from build123d import *

# Parameters (mm, degrees)
EXTRUDE_2_DEPTH              = 40
SKETCH_4_W                   = 2.5
SKETCH_4_H                   = 90
CUT_EXTRUDE_2_DEPTH          = 80
EXTRUDE_3_DEPTH              = 5
FILLET_1_R                   = 10
CHAMFER_1_SIZE               = 10
HOLE_WIZARD_M6_1_D           = 6.6
HOLE_WIZARD_M6_1_CBORE_D     = 11
HOLE_WIZARD_M6_1_CBORE_DEPTH = 6.4
CHAMFER_2_SIZE               = 3
HOLE_WIZARD_7_0_7_1_D        = 7
HOLE_WIZARD_M8_2_D           = 9
HOLE_WIZARD_M8_2_CBORE_D     = 15
HOLE_WIZARD_M8_2_CBORE_DEPTH = 8.6
SKETCH_16_W                  = 163.711624667
SKETCH_16_H                  = 2.5
CUT_EXTRUDE_3_DEPTH          = 179.955301682
SKETCH_17_W                  = 70
SKETCH_17_H                  = 9
CUT_EXTRUDE_4_DEPTH          = 198.834526815
CHAMFER_4_SIZE               = 3
HOLE_WIZARD_7_0_7_2_D        = 7
HOLE_WIZARD_6_0_6_1_D        = 6


with BuildPart() as part:
    # 草图2 → 凸台-拉伸2 (new, symmetric)
    with BuildSketch(Plane.XY):
        Polygon((46, -8.5), (80, -8.5), (80, 8.5), (72, 8.5), (72, 163.5), (56, 163.5), (56, 8.5), (-80, 8.5), (-80, -8.5), (-2, -8.5), (-2, -6.5), (46, -6.5), align=None)
    extrude(amount=EXTRUDE_2_DEPTH, both=True)

    # 草图4 → 切除-拉伸2 (cut)
    with BuildSketch(Plane.ZY.offset(-56)):
        with Locations((-38.75, 53.5)):
            Rectangle(SKETCH_4_W, SKETCH_4_H)
    extrude(amount=-CUT_EXTRUDE_2_DEPTH, mode=Mode.SUBTRACT)

    # 草图5 → 凸台-拉伸3 (add, symmetric)
    with BuildSketch(Plane.XY):
        Polygon((46, 8.5), (6, 8.5), (6, 26.5), (38, 26.5), (38, 83.5), (56, 83.5), (56, 18.5), align=None)
    extrude(amount=EXTRUDE_3_DEPTH, both=True)

    # 圆角1
    fillet_1_edges = [part.edges().sort_by_distance(p)[0] for p in [
        (38, 26.5, 0),
    ]]
    fillet(fillet_1_edges, radius=FILLET_1_R)

    # 倒角1
    chamfer_1_edges = [part.edges().sort_by_distance(p)[0] for p in [
        (6, 26.5, 0),
        (38, 83.5, 0),
    ]]
    chamfer(chamfer_1_edges, length=CHAMFER_1_SIZE)

    # M6 六角凹头螺钉的柱形沉头孔1 (through all)
    with Locations(Plane(origin=(0, 8.5, 0), x_dir=(1, 0, 0), z_dir=(0, 1, 0))):
        with Locations((4.5, 17.5), (39.5, 17.5), (39.5, -17.5), (4.5, -17.5)):
            CounterBoreHole(HOLE_WIZARD_M6_1_D / 2, HOLE_WIZARD_M6_1_CBORE_D / 2, HOLE_WIZARD_M6_1_CBORE_DEPTH)

    # 倒角2
    chamfer_2_edges = [part.edges().sort_by_distance(p)[0] for p in [
        (64, 163.5, 40),
        (64, 163.5, -40),
        (80, 0, -40),
        (-80, 0, 40),
        (80, 0, 40),
    ]]
    chamfer(chamfer_2_edges, length=CHAMFER_2_SIZE)

    # Ø7.0 (7) 直径孔1 (through all)
    with Locations(Plane.ZY.offset(-56)):
        with Locations((-31, 25.5), (-31, 66.5), (31, 66.5), (31, 25.5)):
            Hole(HOLE_WIZARD_7_0_7_1_D / 2)

    # M8 六角凹头螺钉的柱形沉头孔2 (through all)
    with Locations(Plane.ZY.offset(-56)):
        with Locations((-20, 143.5), (-20, 103.5), (20, 103.5), (20, 143.5)):
            CounterBoreHole(HOLE_WIZARD_M8_2_D / 2, HOLE_WIZARD_M8_2_CBORE_D / 2, HOLE_WIZARD_M8_2_CBORE_DEPTH)

    # 草图16 → 切除-拉伸3 (cut, through all)
    with BuildSketch(Plane(origin=(0, 8.5, 0), x_dir=(1, 0, 0), z_dir=(0, 1, 0))):
        with Locations((-1.855812334, 38.75)):
            Rectangle(SKETCH_16_W, SKETCH_16_H)
    extrude(amount=-CUT_EXTRUDE_3_DEPTH, mode=Mode.SUBTRACT)

    # 草图17 → 切除-拉伸4 (cut, through all)
    with BuildSketch(Plane(origin=(0, 0, -37.5), x_dir=(-1, 0, 0), z_dir=(0, 0, -1))):
        with Locations((45, -4)):
            Rectangle(SKETCH_17_W, SKETCH_17_H)
    extrude(amount=-CUT_EXTRUDE_4_DEPTH, mode=Mode.SUBTRACT)

    # 倒角4
    chamfer_4_edges = [part.edges().sort_by_distance(p)[0] for p in [
        (-80, 4.5, -37.5),
    ]]
    chamfer(chamfer_4_edges, length=CHAMFER_4_SIZE)

    # Ø7.0 (7) 直径孔2 (through all)
    with Locations(Plane(origin=(0, 8.5, 0), x_dir=(1, 0, 0), z_dir=(0, 1, 0))):
        with Locations((-28, 15), (-60, 15)):
            Hole(HOLE_WIZARD_7_0_7_2_D / 2)

    # Ø6.0 (6) 直径孔1 (through all)
    with Locations(Plane(origin=(0, 8.5, 0), x_dir=(1, 0, 0), z_dir=(0, 1, 0))):
        with Locations((-70, -31), (-70, -19)):
            Hole(HOLE_WIZARD_6_0_6_1_D / 2)


solid = part.part
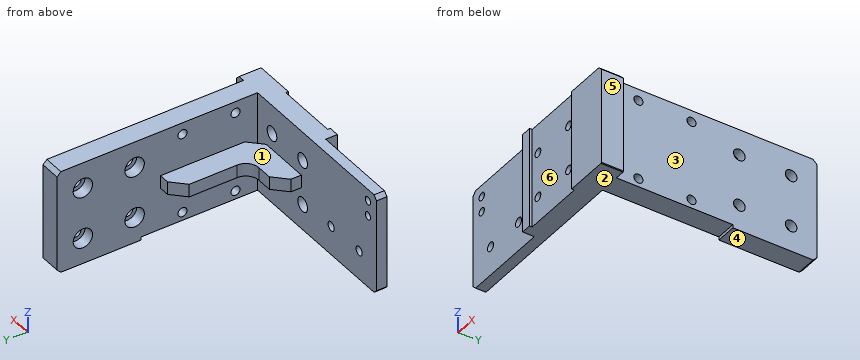
Model file for the job. Use its own axes, mm. Face numbers are marked on the shaded views. A direction names the side the tool comes from. Coordinates: 2 decimals unless noted, no trailing zeros. Order: outer loops, then holes, each group sorted by start corner. A loop starts at its lowest first (then second) coordinate and runs counter-clockwise, first axis right, second up. Notation, with made-up numbers: (-13, 33.5) -> (3, 33.5) arc R5 ccw to (3, 38.5) -> close; hole circle Ø8 at (-2, -2). An arc over 180 degrees is marked (long way). Return JSON: item names as keys, results as strings. Group by question number.
Item 1: Saw through at C-C on z = 31. Write the cut outline in (x, y).
Item 2: Saw through at A-A on x = -70. Write the cut outline in (y, z), then the cut area to 3 significant figures.
Item 3: Wall check: line 1 along Z through (x, y) = (4, 6); line 2 along Y through (x, z) = (58, -20); line 3 along Y through (x, z) = (68.25, -20). Give the ranges that are in metal, low to high. Write a range as [from, to].
Item 4: Saw through at D-D on x = 58.5. State how many separate pieces and enclosed holes the cut face has, then the cut area to 3 significant figures.
Item 5: Flat gauge pins, fed straight in: P1, Ø6.5, axis at x = 51.5, z = 2, coming from the +Y side; P2, Ø2.5, axis at x = 74.5, z = -10, coming from the +Y side; P3, Ø6, axis at y = 80, z = 24, coming from the -X side. Where does each tip first touch, or does it go through?
Item 6: Pull direction X, two halves, no side cores. Call the marked faces 4, 5 and 6: pulls with the +X half, pulls with the -X half, needs draft (parallel to the pull), parting line crosses it, or undercut.
Item 7: Saw through at B-B on y = 103.5. Write the cut outline in (x, z).
Item 8: Tool access for the marked faces 1, 2 and 3: list every direction of +Z, -Z, +X, -X, +Y, -Y with a clear straight run to the whole face (end or side of a thin tool).
Values found:
{
 "1": {"outline": "(-80, 0.5) -> (-73, 0.5) -> (-73, 8.5) -> (-80, 8.5) -> close; (-67, 0.5) -> (-10, 0.5) -> (-10, -8.5) -> (-2, -8.5) -> (-2, -6.5) -> (46, -6.5) -> (46, -8.5) -> (80, -8.5) -> (80, 8.5) -> (72, 8.5) -> (72, 22) -> (56, 22) -> (56, 8.5) -> (-67, 8.5) -> close; (56, 29) -> (72, 29) -> (72, 63) -> (56, 63) -> close; (56, 70) -> (72, 70) -> (72, 163.5) -> (56, 163.5) -> close"},
 "2": {"outline": "(0.5, -37.5) -> (8.5, -37.5) -> (8.5, 16) -> (0.5, 16) -> close; (0.5, 22) -> (8.5, 22) -> (8.5, 28) -> (0.5, 28) -> close; (0.5, 34) -> (8.5, 34) -> (8.5, 40) -> (0.5, 40) -> close", "area": "524 mm2"},
 "3": {"line 1": "z = [-37.5, -22.98], [-12.02, 12.02], [22.98, 40]", "line 2": "y = [-8.5, 96], [111, 136], [151, 163.5]", "line 3": "y = [-8.5, 99], [108, 139], [148, 163.5]"},
 "4": {"separate pieces": "1", "enclosed holes": "8", "area": "12,600 mm2"},
 "5": {"P1": "stops at y = 83.5", "P2": "stops at y = 8.5", "P3": "stops at x = 56"},
 "6": {"face 4": "needs draft", "face 5": "pulls with the +X half", "face 6": "undercut"},
 "7": {"outline": "(56, -40) -> (72, -40) -> (72, -24.5) -> (64.6, -24.5) -> (64.6, -27.5) -> (56, -27.5) -> close; (56, -12.5) -> (64.6, -12.5) -> (64.6, -15.5) -> (72, -15.5) -> (72, 15.5) -> (64.6, 15.5) -> (64.6, 12.5) -> (56, 12.5) -> close; (56, 27.5) -> (64.6, 27.5) -> (64.6, 24.5) -> (72, 24.5) -> (72, 40) -> (56, 40) -> close"},
 "8": {"face 1": "+Z, -X, +Y", "face 2": "-Z, +X, -X, -Y", "face 3": "+Z, -Z, +X, +Y"}
}
